For this review, take the finished solid that the model builds, in its own axes (mm). Face numbers are marked on the shaded views. A direction names the side the tool comes from. Give positions to 0.01 mm unless a question says otherwise; leave off trailing zeros. Order: outer loops, then holes, each group sorted by start corner. A loop starts at its lowest first (then second) coordinate and runs counter-clockwise, first axis right, second up. Notation, with made-up numbers: (88.5, 0) -> (127.5, 0) arc R36 cw to (127.5, 39) -> close; hole circle Ø3 at (22.25, 66). An arc over 180 degrees is marked (long way). Use CSV: the item, a comma, the result in double quotes. Start each with the question number.
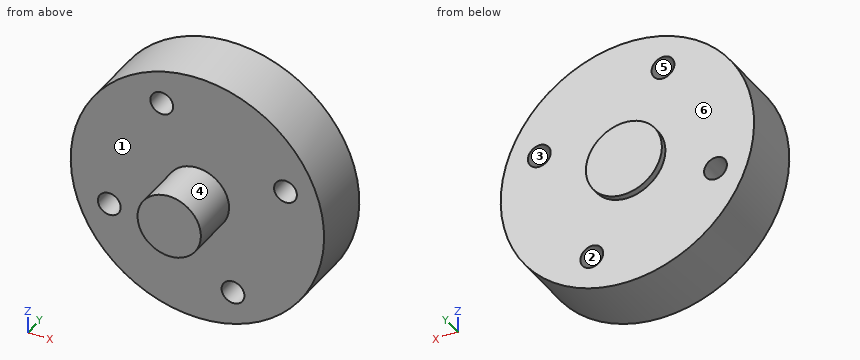
```python
from build123d import *

# Parameters (mm, degrees)
F_18_0_18_DIAMETER_HOLE1_D     = 18
F_18_0_18_DIAMETER_HOLE1_DEPTH = 90


with BuildPart() as part:
    # Sketch1 → Revolve1 (revolve)
    with BuildSketch(Plane.XY, mode=Mode.PRIVATE) as revolve1_sk:
        Polygon((30, -31.6), (100, -31.6), (100, -81.6), (25, -81.6), (25, -121.6), (0, -121.6), (0, -26.6), (30, -26.6), align=None)
    revolve(revolve1_sk.sketch.rotate(Axis((0, 0, 0), (0, 1, 0)), 90), axis=Axis((0, 0, 0), (0, 1, 0)))

    # Ø18.0 (18) Diameter Hole1
    with Locations(Plane(origin=(0, -31.6, 0), x_dir=(1, 0, 0), z_dir=(0, 1, 0))):
        with Locations((-69.533343678, 28.108968621), (-28.108968621, -69.533343678), (69.533343678, -28.108968621), (28.108968621, 69.533343678)):
            Hole(F_18_0_18_DIAMETER_HOLE1_D / 2, depth=F_18_0_18_DIAMETER_HOLE1_DEPTH)


solid = part.part
```
1. Consider section C-C (x = 0). State the section outline as (y, z) points, plus the area to 3 significant figures.
2. For the marked faces 5 and 6, list the 3-axis set-ups (+Z, -Z, +X, -X, +Y, -Y) from which the entire face can be reached by the end or side of a thin tool; tool diameter is ignored.
3. Clearance check with flat-ended pins moving along their axes: P1, Ø1, axis at x = -34, y = -76, coming from the -Z side; P2, Ø3, axis at x = 62, z = 73, coming from the +Y side; P3, Ø6, axis at x = -70.5, z = -66, coming from the -Y side; P4, Ø16, axis at x = 28.11, z = -69.53, coming from the -Y side. State where each tip first meets the part, or that it passes through.
4. Consider section A-A (x = -65). State the section outline as (y, z) points, plus the area to 3 significant figures.
5. Consider section D-D (y = -68). State the section outline as (x, z) points.
6. To check wall thickness, follow L1, parallel to Y at x = 32, z = 36.5; L2, parallel to X at y = -69.5, z = -23; L3, parallel to X at y = -33.5, z = 33.5. State the ranges of each line that lie inside material, in increasing order. Write a range as [from, to].
7. Draft analysis for pull direction Z (two halves, no side actions). For the marked faces 1, 2, 3 and 4, state which applies: +Z half, -Z half, draft (parallel to the pull), parting line (faces both ways), or undercut.
8. Consider section B-B (z = 0). State the section outline as (x, y) points, plus the area to 3 significant figures.
Answer list:
1,outline,"(-121.6, -25) -> (-81.6, -25) -> (-81.6, -100) -> (-31.6, -100) -> (-31.6, -30) -> (-26.6, -30) -> (-26.6, 30) -> (-31.6, 30) -> (-31.6, 100) -> (-81.6, 100) -> (-81.6, 25) -> (-121.6, 25) -> close"
1,area,"12,300 mm2"
2,face 5,"+Y, -Y"
2,face 6,"+Y"
3,P1,"z = -94.22"
3,P2,"y = -31.6"
3,P3,"y = -81.6"
3,P4,"through"
4,outline,"(-81.6, -75.99) -> (-31.6, -75.99) -> (-31.6, -35.88) -> (-81.6, -35.88) -> close; (-81.6, -20.33) -> (-31.6, -20.33) -> (-31.6, 75.99) -> (-81.6, 75.99) -> close"
4,area,"6,820 mm2"
5,outline,"circle Ø200 at (0, 0); hole circle Ø18 at (-69.53, -28.11); hole circle Ø18 at (-28.11, 69.53); hole circle Ø18 at (28.11, -69.53); hole circle Ø18 at (69.53, 28.11)"
6,L1,"[-81.6, -31.6]"
6,L2,"[-97.32, -76.94], [-62.12, 97.32]"
6,L3,"[-94.22, 62.33], [76.74, 94.22]"
7,face 1,"draft"
7,face 2,"undercut"
7,face 3,"undercut"
7,face 4,"parting line"
8,outline,"(-100, -81.6) -> (-25, -81.6) -> (-25, -121.6) -> (25, -121.6) -> (25, -81.6) -> (100, -81.6) -> (100, -31.6) -> (30, -31.6) -> (30, -26.6) -> (-30, -26.6) -> (-30, -31.6) -> (-100, -31.6) -> close"
8,area,"12,300 mm2"
